```python
from build123d import *

# Parameters (mm, degrees)
SKETCH_1_R                   = 60.5
EXTRUDE_2_DEPTH              = 12
CUT_EXTRUDE_START            = 8
SKETCH_3_R                   = 60.5
CUT_EXTRUDE_2_DEPTH          = 339.956913315
SKETCH_5_R                   = 18
CUT_EXTRUDE_3_DEPTH          = 347.956913315
HOLE_WIZARD_M8_1_D           = 9
HOLE_WIZARD_M8_1_CBORE_D     = 15
HOLE_WIZARD_M8_1_CBORE_DEPTH = 9
SKETCH_9_R                   = 5.5
CUT_EXTRUDE_4_DEPTH          = 347.956913315
SKETCH_10_R                  = 60.5
CUT_EXTRUDE_5_DEPTH          = 347.841606064


with BuildPart() as part:
    # 草图1 → 凸台-拉伸2 (new body)
    with BuildSketch(Plane.XY):
        with BuildLine():
            Line((-256, 85.668545552), (256, 85.668545552))
            ThreePointArc((256, 85.668545552), (330.833147735, -22.615725695), (203.084973779, -54.331454448))
            ThreePointArc((203.084973779, -54.331454448), (190.769596292, -46.91488058), (176.627460668, -44.331454448))
            Line((176.627460668, -44.331454448), (-176.627460668, -44.331454448))
            ThreePointArc((-176.627460668, -44.331454448), (-190.769596292, -46.91488058), (-203.084973779, -54.331454448))
            ThreePointArc((-203.084973779, -54.331454448), (-330.833147735, -22.615725695), (-256, 85.668545552))
        make_face()
        with Locations((-256, 5.668545552)):
            Circle(SKETCH_1_R, mode=Mode.SUBTRACT)
        with BuildLine():
            Line((36, 49.668545552), (136, 49.668545552))
            ThreePointArc((136, 49.668545552), (165, 20.668545552), (136, -8.331454448))
            Line((136, -8.331454448), (36, -8.331454448))
            ThreePointArc((36, -8.331454448), (7, 20.668545552), (36, 49.668545552))
        make_face(mode=Mode.SUBTRACT)
        with BuildLine():
            Line((-136, 49.668545552), (-36, 49.668545552))
            ThreePointArc((-36, 49.668545552), (-7, 20.668545552), (-36, -8.331454448))
            Line((-36, -8.331454448), (-136, -8.331454448))
            ThreePointArc((-136, -8.331454448), (-165, 20.668545552), (-136, 49.668545552))
        make_face(mode=Mode.SUBTRACT)
    extrude(amount=EXTRUDE_2_DEPTH)

    # 草图3 → 切除-拉伸2 (cut, through all)
    with BuildSketch(Plane.XY.offset(CUT_EXTRUDE_START)):
        with Locations((256, 5.668545552)):
            Circle(SKETCH_3_R)
    extrude(amount=CUT_EXTRUDE_2_DEPTH, mode=Mode.SUBTRACT)

    # 草图5 → 切除-拉伸3 (cut, through all)
    with BuildSketch(Plane.XY):
        with Locations((256, 5.668545552)):
            Circle(SKETCH_5_R)
    extrude(amount=CUT_EXTRUDE_3_DEPTH, mode=Mode.SUBTRACT)

    # M8 六角圆柱头螺钉的柱形沉头孔1 (through all)
    with Locations(Plane.XY.offset(12)):
        with Locations((-86, 70.668545552), (-86, -29.331454448), (86, 70.668545552), (86, -29.331454448)):
            CounterBoreHole(HOLE_WIZARD_M8_1_D / 2, HOLE_WIZARD_M8_1_CBORE_D / 2, HOLE_WIZARD_M8_1_CBORE_DEPTH)

    # 草图9 → 切除-拉伸4 (cut, through all)
    with BuildSketch(Plane(origin=(0, 0, 0), x_dir=(-1, 0, 0), z_dir=(0, 0, -1))):
        with Locations((256, 75.918545552)):
            Circle(SKETCH_9_R)
        with Locations((326.25, 5.668545552)):
            Circle(SKETCH_9_R)
        with Locations((256, -64.581454448)):
            Circle(SKETCH_9_R)
        with Locations((185.75, 5.668545552)):
            Circle(SKETCH_9_R)
    extrude(amount=-CUT_EXTRUDE_4_DEPTH, mode=Mode.SUBTRACT)

    # 草图10 → 切除-拉伸5 (cut, through all)
    with BuildSketch(Plane.XY.offset(8)):
        with Locations((256, 5.668545552)):
            Circle(SKETCH_10_R)
    extrude(amount=-CUT_EXTRUDE_5_DEPTH, mode=Mode.SUBTRACT)


solid = part.part
```
CAD build for the part. Positions are in the model's coordinates, mm. A direction names the side the tool comes from. Give positions to 0.01 mm unless a question says otherwise; leave off trailing zeros. Order: outer loops, then holes, each group sorted by start corner. A loop starts at its lowest first (then second) coordinate and runs counter-clockwise, first axis right, second up. Notation, with made-up numbers: M 54.5,82.5 L 97.5,82.5 A18 ccw 97.5,106.5 Z; hole C 57.25,-12.5 d5. An arc over 180 degrees is marked long. Put each result on its own line as item: value. Start each with the question number.
(1) Mould opens along X. For faces 4 (the flat face through (5, 25, 0)), 5 (the cylindrical face through (7.007, 20.031, 5.916)) say: +X half, -X half, draft (parallel to the pull), parting line (faces both ways), or undercut.
(2) Drill centre lines: line 1 along Y through (x, z) = (86, 7.25); line 2 along Y through (x, z) = (-86, 1.4); line 3 along X through (y, z) = (13.5, 6). Where is each one in solid material? Low to high.
(3) Saw through at D-D, the plane x = -212. Write the cut outline in (y, z), then the cut area to 3 significant figures.
(4) Saw through at A-A, the plane x = -49. Write the cut outline in (y, z), then the cut area to 3 significant figures.
(5) Saw through at C-C, the plane z = 8. Give the number of separate pieces and of enclosed holes in the cut face, then the cut area to 3 significant figures.
(6) Saw through at B-B, the plane y = 38. Write the cut outline in (x, z).
(7) Which spindle directions (+Z, -Z, +X, -X, +Y, -Y) get a long thin tool onto all of the face, cutting with end or side? Do faces 1 (the cylindrical face through (-91.528, 75.737, 7.563)), 2 (the flat face through (-87, 49.669, 6)), 3 (the cylindrical face through (190.959, -46.987, 5.916)). Say none if no direction does.
(8) Flat gauge pins, fed straight in: pin 1 Ø10.5 at (x, y) = (86, -29.33) entering from +Z; pin 2 Ø3.5 at (x, z) = (-8, 5) entering from -Y; pin 3 Ø12.5 at (x, y) = (-185.75, 5.67) entering from +Z; pin 4 Ø5.5 at (x, y) = (86, 70.67) entering from -Z. Where does each tip first touch, or does it go through?
Check result:
1. face 4: draft
1. face 5: undercut
2. line 1: y = -44.33 to -36.83, -21.83 to -8.33, 49.67 to 63.17, 78.17 to 85.67
2. line 2: y = -44.33 to -33.83, -24.83 to -8.33, 49.67 to 66.17, 75.17 to 85.67
2. line 3: x = -335.62 to -315.99, -196.01 to -164.1, -7.9 to 7.9, 164.1 to 196.01, 315.99 to 335.62
3. outline: M -61.14,0 L -35.86,0 L -35.86,12 L -61.14,12 Z; M 47.19,0 L 85.67,0 L 85.67,12 L 47.19,12 Z
3. area: 765 mm2
4. outline: M -44.33,0 L -8.33,0 L -8.33,12 L -44.33,12 Z; M 49.67,0 L 85.67,0 L 85.67,12 L 49.67,12 Z
4. area: 864 mm2
5. separate pieces: 1
5. enclosed holes: 12
5. area: 48,400 mm2
6. outline: M -329.18,0 L -307.14,0 L -307.14,12 L -329.18,12 Z; M -204.86,0 L -159.25,0 L -159.25,12 L -204.86,12 Z; M -12.75,0 L 12.75,0 L 12.75,12 L -12.75,12 Z; M 159.25,0 L 204.86,0 L 204.86,12 L 159.25,12 Z; M 307.14,0 L 329.18,0 L 329.18,12 L 307.14,12 Z
7. face 1: +Z
7. face 2: +Z, -Z
7. face 3: +Z, -Z, -Y
8. pin 1: stops at z = 3
8. pin 2: stops at y = -44.33
8. pin 3: stops at z = 12
8. pin 4: passes through
